```python
from build123d import *

# Parameters (mm, degrees)
SKETCH2_R = 3.25


with BuildPart() as part:
    # Sweep1: sweep along a path in Sketch1
    with BuildLine(Plane.XY) as sweep1_path:
        Line((0, 0), (0, 1173))
        ThreePointArc((0, 1173), (12.30151519, 1202.69848481), (42, 1215))
        Line((42, 1215), (1580, 1215))
        ThreePointArc((1580, 1215), (1609.69848481, 1202.69848481), (1622, 1173))
        Line((1622, 1173), (1622, 985))
    # Sketch2 → Sweep1 (sweep)
    with BuildSketch(Plane(origin=(0, 0, 0), x_dir=(1, 0, 0), z_dir=(0, 1, 0))):
        Circle(SKETCH2_R)
    sweep(path=sweep1_path.line)


solid = part.part
```
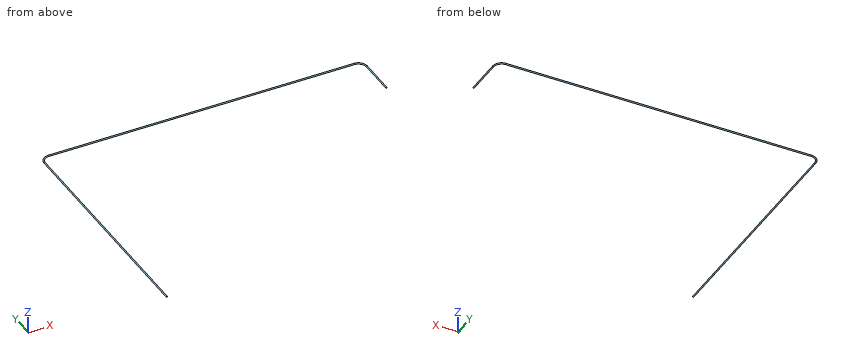
Here's how the part is built. I have some questions about the finished solid (model axes, mm). Coordinates: 2 decimals unless noted, no trailing zeros. Write each loop counter-clockwise with the first axis right and the second up, starting at its lowest first coordinate (ties: lowest second). Pieces come first, ordered by that corner, then holes. Notation, with made-up numbers: (9.5, 28.25) -> (41.5, 28.25) arc R23 cw to (41.5, 54.25) -> close; hole circle Ø4 at (57, -22.5). An arc over 180 degrees is marked (long way). Use a Markdown table: item, result. Add a question column.
(1) I'm going to push flat-ended pins straight in: P1, Ø1, axis at x = 1034, z = -2.5, coming from the -Y side; P2, Ø2, axis at x = 1620.5, z = 0.5, coming from the -Y side. Where does each tip first touch, or does it pass through?
(2) Please list where these lines run through material, in increasing order: line 1 (X direction, y = 1001.5, z = 1.25); line 2 (X direction, y = 423.5, z = 1.25); line 3 (X direction, y = 629, z = 0.75).
(3) If we section it at A-A, the plane y = 1093.5: Write out the boundary of the cut face in (x, z).
(4) If we section it at C-C, the plane x = 1195: Write out the boundary of the cut face in (y, z), and give its area (3 significant figures).
(5) If we section it at D-D, the plane y = 739.5: Write out the boundary of the cut face in (x, z).
(6) If we section it at B-B, the plane z = 0: Write out the boundary of the cut face in (x, y), and give its area (3 significant figures).
Outcome:
| question | item | result |
|---|---|---|
| 1 | P1 | stops at y = 1212.44 |
| 1 | P2 | stops at y = 985 |
| 2 | line 1 | x = -3 to 3, 1619 to 1625 |
| 2 | line 2 | x = -3 to 3 |
| 2 | line 3 | x = -3.16 to 3.16 |
| 3 | outline | circle Ø6.5 at (0, 0); circle Ø6.5 at (1622, 0) |
| 4 | outline | circle Ø6.5 at (1215, 0) |
| 4 | area | 33.2 mm^2 |
| 5 | outline | circle Ø6.5 at (0, 0) |
| 6 | outline | (-3.25, 0) -> (3.25, 0) -> (3.25, 1173) arc R38.75 cw to (42, 1211.75) -> (1580, 1211.75) arc R38.75 cw to (1618.75, 1173) -> (1618.75, 985) -> (1625.25, 985) -> (1625.25, 1173) arc R45.25 ccw to (1580, 1218.25) -> (42, 1218.25) arc R45.25 ccw to (-3.25, 1173) -> close |
| 6 | area | 19,700 mm^2 |
